Input: part model. Units: mm. Frame: model coordinates. Face numbers are marked on the shaded views. Give positions to 0.01 mm unless a question says otherwise; leave off trailing zeros. Order: outer loops, then holes, each group sorted by start corner. A loop starts at its lowest first (then second) coordinate and runs counter-clockwise, first axis right, second up. Notation, with made-up numbers: M 40,-11 L 58,-11 A16 cw 58,-6 Z; hole C -20,4 d4. An arc over 180 degrees is marked long. Use a Markdown table: item, result.
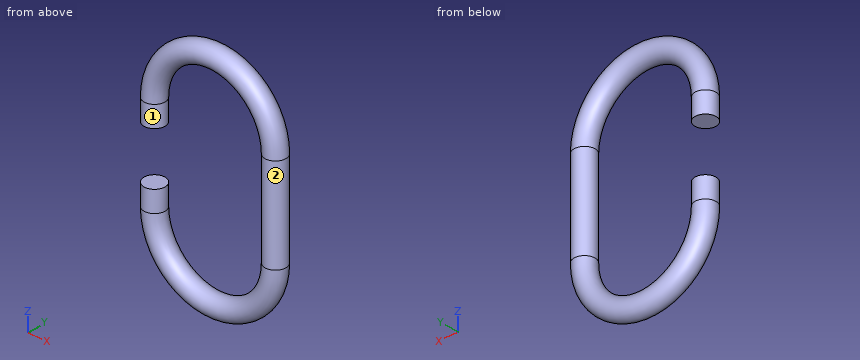
from build123d import *

# Parameters (mm, degrees)
SKETCH2_R = 4


with BuildPart() as part:
    # Sweep1: sweep along a path in Sketch1
    with BuildLine(Plane(origin=(0, 0, 0), x_dir=(1, 0, 0), z_dir=(0, 1, 0))) as sweep1_path:
        Line((-23, 10), (-23, 18))
        ThreePointArc((-23, 18), (0, 41), (23, 18))
        Line((23, 18), (23, -18))
        ThreePointArc((23, -18), (0, -41), (-23, -18))
        Line((-23, -18), (-23, -10))
    # Sketch2 → Sweep1 (sweep)
    with BuildSketch(Plane.XY.offset(-10)):
        with Locations((-23, 0)):
            Circle(SKETCH2_R)
    sweep(path=sweep1_path.line)


solid = part.part
1) Material intervals for line 1 (X direction, y = 0.5, z = 32.5); line 2 (X direction, y = 0.75, z = 35.5); line 3 (Z direction, x = 4, y = 1.75), sorted ascending. Write a range as from..to.
Response values:
| item | result |
|---|---|
| line 1 | x = -22.74..-12.33, 12.33..22.74 |
| line 2 | x = -20.47..-7.58, 7.58..20.47 |
| line 3 | z = -44.29..-36.99, 36.99..44.29 |
2) Cut plane A-A on z = 13.5. Return loops of the section in (x, y).
Response values:
| item | result |
|---|---|
| outline | C -23,0 d8; C 23,0 d8 |
3) First-contact query: pin 1 Ø4 at (x, y) = (-24.5, -1.5) entering from -Z; pin 2 Ø1.5 at (y, z) = (2, -31.5) entering from -X; pin 3 Ø3 at (x, z) = (18.5, 1) entering from -Y; pin 4 Ø10 at (x, z) = (12, 33.5) entering from +Y. Flat tips, straight axial feed; report the tip coordinate or a pass-through.
Response values:
| item | result |
|---|---|
| pin 1 | stops at z = -32.6 |
| pin 2 | stops at x = -23.36 |
| pin 3 | stops at y = -2.65 |
| pin 4 | stops at y = 4 |
4) Mould query, pull axis X, two halves, no side actions, for the marked faces 1 and 2. Classes: released by +X, released by -X, zero draft, split by the parting line, or undercut.
Response values:
| item | result |
|---|---|
| face 1 | undercut |
| face 2 | undercut |
5) Cut plane B-B on y = -1.5. Return loops of the section in (x, z).
Response values:
| item | result |
|---|---|
| outline | M -26.71,-18 A26.71 ccw 26.71,-18 L 26.71,18 A26.71 ccw -26.71,18 L -26.71,10 L -19.29,10 L -19.29,18 A19.29 cw 19.29,18 L 19.29,-18 A19.29 cw -19.29,-18 L -19.29,-10 L -26.71,-10 Z |
